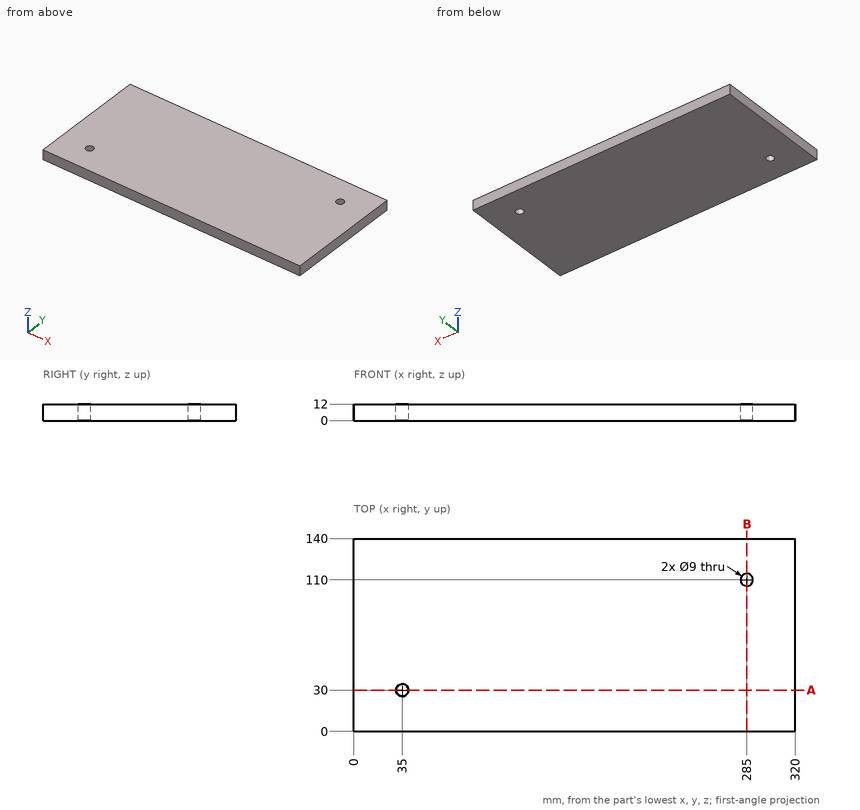
Here's the drawing with two shaded views (mm, measured from the low corner). I have some questions. Coordinates: 2 decimals unless noted, no trailing zeros. Loops run counter-clockwise (first coordinate to the right, second up) from the corner with the lowest first, then second, coordinate; pieces in that order, holes last. Notation, with made-up numbers: M 87.25,64 L 110.25,64 A27 cw 110.25,96 Z; hole C 86.5,58.5 d10. An arc over 180 degrees is marked long. Answer as CSV lines item,"result". Start each with the question number.
1. Suppose I cut it at A-A, the plane y = 30. List the corners of the cut face in (x, z) for me, plus the area to 3 significant figures.
2. Suppose I cut it at B-B, the plane x = 285. List the corners of the cut face in (y, z) for me, plus the area to 3 significant figures.
3. For pin 1 Ø1.5 at (x, z) = (53.5, 2.5) entering from -Y, with a flat end and sliding along its axis, tell me the tip position at first contact or that it passes through.
4. If I drill on probe 1 along X at (y, z) = (30, 9.5); probe 2 along Y at (x, z) = (35, 2.5); probe 3 along Y at (x, z) = (285, 8.75), over which ranges is the centre line in solid material (lowest first)? Write a range as [from, to].
Output:
1,outline,"M 0,0 L 30.5,0 L 30.5,12 L 0,12 Z; M 39.5,0 L 320,0 L 320,12 L 39.5,12 Z"
1,area,"3,730 mm^2"
2,outline,"M 0,0 L 105.5,0 L 105.5,12 L 0,12 Z; M 114.5,0 L 140,0 L 140,12 L 114.5,12 Z"
2,area,"1,570 mm^2"
3,pin 1,"stops at y = 0"
4,probe 1,"x = [0, 30.5], [39.5, 320]"
4,probe 2,"y = [0, 25.5], [34.5, 140]"
4,probe 3,"y = [0, 105.5], [114.5, 140]"
